Read the model definition and answer for the solid it produces. Units are mm, in the model's axes. A direction names the side the tool comes from. Round coordinates to 2 decimals unless told otherwise and drop trailing zeros. Order: outer loops, then holes, each group sorted by start corner. A loop starts at its lowest first (then second) coordinate and runs counter-clockwise, first axis right, second up. Notation, with made-up numbers: (-22, 71.5) -> (32, 71.5) arc R23 cw to (32, 87.5) -> close; hole circle Ø5 at (29.25, 63.5). An arc over 180 degrees is marked (long way). One line per item, written item: value. Start each with the question number.
1. Section D-D (x = 6) is taken. Give the vertices of the cut face in (y, z).
2. Section A-A (z = 20) is taken. Give the vertices of the cut face in (x, y), then the cut area to 3 significant figures.
3. Section B-B (y = 56) is taken. Give the vertices of the cut face in (x, z), then the cut area to 3 significant figures.
4. The mould has two halves that part along X. Classify faces 1 (the face through (41, 26, -1)), 2 (the face through (-30, 46, 45)), 3 (the face through (-30.15, 78.88, 18.18)): released by +X, released by -X, zero draft, split by the parting line, or undercut.
5. For faces 4 (the face through (-28, 54, -59)), 5 (the face through (0, 32, -47)), 6 (the face through (-29, 22, -29)), determine the directions among +Z, -Z, +X, -X, +Y, -Y from which every point of the face is accessible in a straight line to the end or side of a thin tool.
6. Flat-ended cylindrical pins translate along their axes: pin 1 Ø1.5 at (x, y) = (-5, 14.5) entering from +Z; pin 2 Ø18.5 at (x, y) = (31, 14.5) entering from +Z; pin 3 Ø3.5 at (x, z) = (-35.5, -27.5) entering from +Y. Find the tip coordinate at first contact, or state that the pin passes through.
7. Section C-C (x = 27) is taken. Give the vertices of the cut face in (y, z).
8. Consider line 1 (X direction, y = 23.5, z = 21); line 2 (Y direction, x = -34, z = 20); line 3 (Z direction, x = 30.5, y = 45.5). Determine where each line is inside the solid, lowest interval first.
from build123d import *

# Parameters (mm, degrees)
BASE_PLATE_DEPTH            = 15
RAISED_WALL_DEPTH           = 15
PIVOT_LUG_DEPTH             = 22
LUG_START                   = -22
LUG_EXTENSION_DEPTH         = 22
PIVOT_BORE_SKETCH_R         = 14
PIVOT_BORE_DEPTH            = 106
BEARING_BLOCK_DEPTH         = 82
BEARING_BOSS_DEPTH          = 28
BEARING_SEAT_CUT_DEPTH      = 44
BASE_MOUNTING_HOLE_SKETCH_R = 11
BASE_MOUNTING_HOLE_DEPTH    = 44


with BuildPart() as part:
    # Base Plate Sketch → Base Plate (new body)
    with BuildSketch(Plane(origin=(0, 0, 0), x_dir=(1, 0, 0), z_dir=(0, 1, 0))):
        with BuildLine():
            Line((18, -70), (41, -70))
            Line((41, -70), (41, 0))
            Line((41, 0), (41, 70))
            Line((41, 70), (-41, 70))
            Line((-41, 70), (-41, -70))
            Line((-41, -70), (-18, -70))
            ThreePointArc((-18, -70), (0, -88), (18, -70))
        make_face()
    extrude(amount=BASE_PLATE_DEPTH)

    # Raised Wall Sketch → Raised Wall (add)
    with BuildSketch(Plane(origin=(0, 15, 0), x_dir=(1, 0, 0), z_dir=(0, 1, 0))):
        Polygon((41, -70), (29, -70), (29, 52), (-29, 52), (-29, -70), (-41, -70), (-41, 70), (41, 70), align=None)
    extrude(amount=RAISED_WALL_DEPTH)

    # Pivot Lug Sketch → Pivot Lug (add)
    with BuildSketch(Plane.ZY.offset(41)):
        with BuildLine():
            Line((45, 30), (45, 15))
            Line((45, 15), (-5, 15))
            Line((-5, 15), (-5, 30))
            Line((-5, 30), (-5, 65))
            ThreePointArc((-5, 65), (20, 90), (45, 65))
            Line((45, 65), (45, 30))
        make_face()
    extrude(amount=-PIVOT_LUG_DEPTH)

    # Lug Extension Sketch → Lug Extension (add)
    with BuildSketch(Plane(origin=(41, 0, 0), x_dir=(0, 0, -1), z_dir=(1, 0, 0)).offset(LUG_START)):
        with BuildLine():
            Line((5, 15), (-20, 15))
            Line((-20, 15), (-45, 15))
            Line((-45, 15), (-45, 65))
            ThreePointArc((-45, 65), (-20, 90), (5, 65))
            Line((5, 65), (5, 15))
        make_face()
    extrude(amount=LUG_EXTENSION_DEPTH)

    # Pivot Bore Sketch → Pivot Bore (cut)
    with BuildSketch(Plane.ZY.offset(41)):
        with Locations((20, 65)):
            Circle(PIVOT_BORE_SKETCH_R)
    extrude(amount=-PIVOT_BORE_DEPTH, mode=Mode.SUBTRACT)

    # Bearing Block Sketch → Bearing Block (add)
    with BuildSketch(Plane.ZY.offset(41)):
        Polygon((-70, 0), (-70, 54), (-52, 54), (-52, 30), (-52, 0), align=None)
    extrude(amount=-BEARING_BLOCK_DEPTH)

    # Bearing Boss Sketch → Bearing Boss (add)
    with BuildSketch(Plane(origin=(0, 0, -70), x_dir=(-1, 0, 0), z_dir=(0, 0, -1))):
        with BuildLine():
            Line((-22, 54), (22, 54))
            ThreePointArc((22, 54), (0, 32), (-22, 54))
        make_face()
    extrude(amount=-BEARING_BOSS_DEPTH)

    # Bearing Seat Sketch → Bearing Seat Cut (cut)
    with BuildSketch(Plane(origin=(0, 0, -70), x_dir=(-1, 0, 0), z_dir=(0, 0, -1))):
        with BuildLine():
            Line((-14, 54), (14, 54))
            ThreePointArc((14, 54), (0, 40), (-14, 54))
        make_face()
    extrude(amount=-BEARING_SEAT_CUT_DEPTH, mode=Mode.SUBTRACT)

    # Base Mounting Hole Sketch → Base Mounting Hole (cut)
    with BuildSketch(Plane(origin=(0, 15, 0), x_dir=(1, 0, 0), z_dir=(0, 1, 0))):
        with Locations(Location((0, -70, 0), (0, 0, 270))):
            Circle(BASE_MOUNTING_HOLE_SKETCH_R)
    extrude(amount=-BASE_MOUNTING_HOLE_DEPTH, mode=Mode.SUBTRACT)


solid = part.part
Answer:
1. outline: (0, -70) -> (41.35, -70) -> (41.35, -42) -> (32.83, -42) -> (32.83, -52) -> (15, -52) -> (15, 60.78) -> (0, 60.78) -> close; (0, 79.22) -> (15, 79.22) -> (15, 86.97) -> (0, 86.97) -> close
2. outline: (-41, 0) -> (41, 0) -> (41, 51) -> (19, 51) -> (19, 15) -> (-19, 15) -> (-19, 51) -> (-41, 51) -> close; (-41, 79) -> (-19, 79) -> (-19, 90) -> (-41, 90) -> close; (19, 79) -> (41, 79) -> (41, 90) -> (19, 90) -> close
2. area: 3,300 mm^2
3. outline: (-41, -5) -> (-19, -5) -> (-19, 9.28) -> (-41, 9.28) -> close; (-41, 30.72) -> (-19, 30.72) -> (-19, 45) -> (-41, 45) -> close; (19, -5) -> (41, -5) -> (41, 9.28) -> (19, 9.28) -> close; (19, 30.72) -> (41, 30.72) -> (41, 45) -> (19, 45) -> close
3. area: 1,260 mm^2
4. face 1: released by +X
4. face 2: undercut
4. face 3: zero draft
5. face 4: -Z, +X, -X, +Y
5. face 5: none
5. face 6: +Y
6. pin 1: z = 87.49
6. pin 2: z = 70
6. pin 3: y = 30
7. outline: (0, -70) -> (54, -70) -> (54, -52) -> (15, -52) -> (15, -5) -> (65, -5) arc R25 ccw to (65, 45) -> (15, 45) -> (15, 70) -> (0, 70) -> close; hole circle Ø28 at (65, 20)
8. line 1: -41 to -19, 19 to 41
8. line 2: 0 to 51, 79 to 90
8. line 3: -70 to -52, -5 to 45
